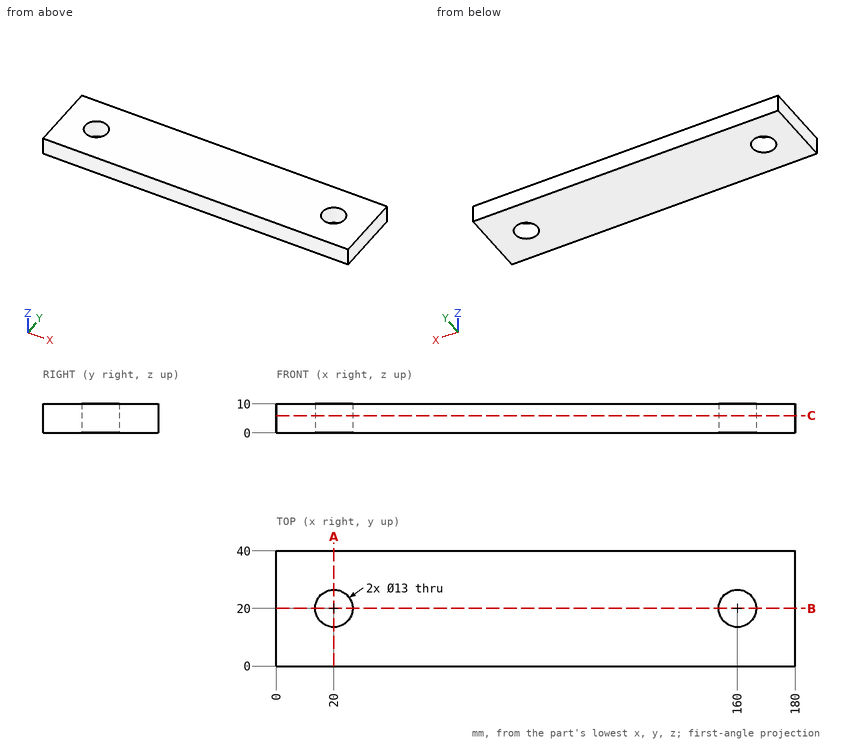
Study the drawing (mm; zero at the part's minimum x, y, z) and answer. Coordinates: 2 decimals unless noted, no trailing zeros. Write each loop counter-clockwise with the first axis right and the second up, starting at its lowest first coordinate (ties: lowest second). Pieces come first, ordered by that corner, then holes. Notation, with made-up numbers: (-23.75, -10.75) - (29.25, -10.75) arc R21 cw to (29.25, 5.25) - close; hole circle Ø1 at (-30, -10). An arc over 180 degrees is marked (long way). Answer as a JSON object with one key per item and string values. Group by question number.
1. A cutting plane is placed at A-A (x = 20). Determine the outline of the cut face in (y, z), plus the area to 3 significant figures.
2. Consider L1, parallel to X at y = 19.5, z = 7; L2, parallel to Y at x = 20, z = 3; L3, parallel to X at y = 25, z = 4. Determine where each line is inside the solid, lowest interval first. Write a range as [from, to].
3. A cutting plane is placed at C-C (z = 6). Determine the outline of the cut face in (x, y), plus the area to 3 significant figures.
4. A cutting plane is placed at B-B (y = 20). Determine the outline of the cut face in (x, z).
5. Each of these flat-tipped pins is pushed along its axis until it touches: P1, Ø11.5, axis at x = 20, y = 20, coming from the +Z side; P2, Ø21, axis at x = 160, y = 20, coming from the +Z side. Where does it stop, or does it pass through?
Worked out:
{
 "1": {"outline": "(0, 0) - (13.5, 0) - (13.5, 10) - (0, 10) - close; (26.5, 0) - (40, 0) - (40, 10) - (26.5, 10) - close", "area": "270 mm²"},
 "2": {"L1": "x = [0, 13.52], [26.48, 153.52], [166.48, 180]", "L2": "y = [0, 13.5], [26.5, 40]", "L3": "x = [0, 15.85], [24.15, 155.85], [164.15, 180]"},
 "3": {"outline": "(0, 0) - (180, 0) - (180, 40) - (0, 40) - close; hole circle Ø13 at (20, 20); hole circle Ø13 at (160, 20)", "area": "6,930 mm²"},
 "4": {"outline": "(0, 0) - (13.5, 0) - (13.5, 10) - (0, 10) - close; (26.5, 0) - (153.5, 0) - (153.5, 10) - (26.5, 10) - close; (166.5, 0) - (180, 0) - (180, 10) - (166.5, 10) - close"},
 "5": {"P1": "passes through", "P2": "stops at z = 10"}
}
